Check sheet for the modelled part. Datum: model origin and axes. Units: mm. A direction names the side the tool comes from. Round coordinates to 2 decimals unless told otherwise and drop trailing zeros. Write each loop counter-clockwise with the first axis right and the second up, starting at its lowest first coordinate (ties: lowest second). Pieces come first, ordered by that corner, then holes.
Item 1: Cross-section at C-C on y = -120. Enter the section's corners in (x, z).
Item 2: Cross-section at B-B on x = -10. Enter the section's corners in (y, z), plus the area to 4 significant figures.
Item 3: Cross-section at A-A on z = 20.5. Enter the section's corners in (x, y), plus the area to 3 significant figures.
Item 4: Cross-section at D-D on x = 22.5. Enter the section's corners in (y, z).
Item 5: Material ranges on line 1 (Y direction, x = 5, z = 1.05); line 2 (X direction, y = -86, z = 12); line 3 (Y direction, x = 20, z = 5.75), recorded low to high.
Item 6: Tool access check on faces 1 (the flat face through (22, -93, 7)), 2 (the flat face through (34, -88, 12)), 3 (the flat face through (22, -25, 7)), 4 (the flat face through (-17.5, -47, 9)). Record the directions out of +Z, -Z, +X, -X, +Y, -Y that give a thin tool (end or side, any length) a straight path to the whole face; none if there is none.
Item 7: Release check for a two-part mould opening along X. For faces 5 (the flat face through (34, -30, 12)), 6 (the flat face through (22, -83, 7)), 7 (the cylindrical face through (18.064, -87.93, 14.807)), 8 (the cylindrical face through (-9.84, -47.48, 23.5)) record: +X half, -X half, draft (parallel to the pull), parting line (faces both ways), or undercut.
Item 8: Go/stop test with flat-tipped pins: pin 1 Ø0.9 at (y, z) = (-48, 6.5) entering from -X; pin 2 Ø10 at (x, z) = (27, 9.5) entering from -Y; pin 3 Ø2 at (x, z) = (30, 7) entering from +Y; pin 4 Ø3.5 at (x, z) = (-10, 16) entering from +Y. Record where each tip stops, or that it passes through.
from build123d import *

# Parameters (mm, degrees)
SKETCH_1_R             = 3
EXTRUDE_1_DEPTH        = 2
EXTRUDE_START          = -25
SKETCH_2_W             = 23
SKETCH_2_H             = 20
SKETCH_2_R             = 5
EXTRUDE_2_DEPTH        = 10
PATTERN_LINEAR_1_COUNT = 2
PATTERN_LINEAR_1_PITCH = 58
EXTRUDE_START_2        = -11
SKETCH_3_R             = 2
EXTRUDE_3_DEPTH        = 3


with BuildPart() as part:
    # 草图1 → 凸台-拉伸1 (new body)
    with BuildSketch(Plane.XY):
        Polygon((0, 0), (45, 0), (45, -25), (35, -25), (35, -130), (10, -130), (10, -60), (-25, -60), (-25, -35), (10, -35), (10, -25), (0, -25), align=None)
        with Locations((5, -5)):
            Circle(SKETCH_1_R, mode=Mode.SUBTRACT)
        with Locations((40, -5)):
            Circle(SKETCH_1_R, mode=Mode.SUBTRACT)
        with Locations((5, -20)):
            Circle(SKETCH_1_R, mode=Mode.SUBTRACT)
        with Locations((40, -20)):
            Circle(SKETCH_1_R, mode=Mode.SUBTRACT)
        with Locations((16.5, -120)):
            Circle(SKETCH_1_R, mode=Mode.SUBTRACT)
        with Locations((28.5, -120)):
            Circle(SKETCH_1_R, mode=Mode.SUBTRACT)
    extrude(amount=EXTRUDE_1_DEPTH)

    # 草图2 → 凸台-拉伸2 (add)
    with BuildSketch(Plane(origin=(0, 0, 0), x_dir=(1, 0, 0), z_dir=(0, 1, 0)).offset(EXTRUDE_START)):
        with Locations((22.5, -12)):
            Rectangle(SKETCH_2_W, SKETCH_2_H)
        with Locations(Location((22.5, -12.5, 0), (0, 0, 270))):
            Circle(SKETCH_2_R, mode=Mode.SUBTRACT)
    extrude_2 = extrude(amount=-EXTRUDE_2_DEPTH)

    # 阵列(线性)1: 凸台-拉伸2 ×2
    with Locations(*[(0, -i * PATTERN_LINEAR_1_PITCH, 0) for i in range(1, PATTERN_LINEAR_1_COUNT)]):
        add(extrude_2)

    # 草图3 → 凸台-拉伸3 (add)
    with BuildSketch(Plane(origin=(0, -35, 0), x_dir=(1, 0, 0), z_dir=(0, 1, 0)).offset(EXTRUDE_START_2)):
        with BuildLine():
            Line((-17.5, -2), (-2.5, -2))
            Line((-2.5, -2), (-2.5, -16))
            ThreePointArc((-2.5, -16), (-10, -23.5), (-17.5, -16))
            Line((-17.5, -16), (-17.5, -2))
        make_face()
        with Locations(Location((-10, -16, 0), (0, 0, 270))):
            Circle(SKETCH_3_R, mode=Mode.SUBTRACT)
    extrude(amount=-EXTRUDE_3_DEPTH)


solid = part.part
Response values:
1. outline: (10, 0) - (13.5, 0) - (13.5, 2) - (10, 2) - close; (19.5, 0) - (25.5, 0) - (25.5, 2) - (19.5, 2) - close; (31.5, 0) - (35, 0) - (35, 2) - (31.5, 2) - close
2. outline: (-60, 0) - (-35, 0) - (-35, 2) - (-46, 2) - (-46, 14) - (-49, 14) - (-49, 2) - (-60, 2) - close; (-49, 18) - (-46, 18) - (-46, 23.5) - (-49, 23.5) - close
2. area: 102.5 mm2
3. outline: (-16, -49) - (-4, -49) - (-4, -46) - (-16, -46) - close; (11, -93) - (34, -93) - (34, -83) - (11, -83) - close; (11, -35) - (34, -35) - (34, -25) - (11, -25) - close
3. area: 496 mm2
4. outline: (-130, 0) - (0, 0) - (0, 2) - (-25, 2) - (-25, 7.5) - (-35, 7.5) - (-35, 2) - (-83, 2) - (-83, 7.5) - (-93, 7.5) - (-93, 2) - (-130, 2) - close; (-93, 17.5) - (-83, 17.5) - (-83, 22) - (-93, 22) - close; (-35, 17.5) - (-25, 17.5) - (-25, 22) - (-35, 22) - close
5. line 1: y = -60 to -35, -25 to -23, -17 to -8, -2 to 0
5. line 2: x = 11 to 17.53, 27.47 to 34
5. line 3: y = -93 to -83, -35 to -25
6. face 1: +Z, +X, -X, -Y
6. face 2: +Z, +X, +Y, -Y
6. face 3: +Z, +X, -X, +Y
6. face 4: +Z, -X, +Y, -Y
7. face 5: +X half
7. face 6: draft
7. face 7: undercut
7. face 8: parting line
8. pin 1: stops at x = -17.5
8. pin 2: stops at y = -93
8. pin 3: stops at y = -25
8. pin 4: passes through
